The listing builds one solid part. Answer for the finished solid, in the listing's coordinates (mm). A direction names the side the tool comes from. Coordinates: 2 decimals unless noted, no trailing zeros. Write each loop counter-clockwise with the first axis right and the second up, starting at its lowest first coordinate (ties: lowest second). Pieces come first, ordered by that corner, then holes. Notation, with made-up numbers: M 6,31 L 37,31 A16 ccw 37,37 Z; hole C 42.25,89.25 d6. An arc over 180 degrees is marked long. Answer as CSV lines item,"result". Start each with the question number.
```python
from build123d import *


with BuildPart() as part:
    # 草图1 → 旋转1 (revolve)
    with BuildSketch(Plane.XY, mode=Mode.PRIVATE) as revolve_1_sk:
        with BuildLine():
            Line((0, 0), (0, 12.5))
            Line((0, 12.5), (1, 13.5))
            Line((1, 13.5), (41, 13.5))
            Line((41, 13.5), (41, 12.5))
            Line((41, 12.5), (45, 12.5))
            Line((45, 12.5), (45, 13))
            ThreePointArc((45, 13), (45.878679656, 15.121320344), (48, 16))
            Line((48, 16), (711, 16))
            Line((711, 16), (711, 14.5))
            Line((711, 14.5), (713, 14.5))
            Line((713, 14.5), (713, 16))
            Line((713, 16), (718, 16))
            Line((718, 16), (718, 14.5))
            Line((718, 14.5), (720, 14.5))
            Line((720, 14.5), (720, 16))
            Line((720, 16), (724, 16))
            Line((724, 16), (725, 15))
            Line((725, 15), (725, 10))
            Line((725, 10), (754, 10))
            Line((754, 10), (755, 9))
            Line((755, 9), (755, 0))
            Line((755, 0), (0, 0))
        make_face()
    revolve(revolve_1_sk.sketch.rotate(Axis((0, 0, 0), (1, 0, 0)), 90), axis=Axis((0, 0, 0), (1, 0, 0)))


solid = part.part
```
1) For a pull along X with two mould halves and no side action, classify faces 4 (the face through (384.14, 15.62, -3.47)), 5 (the face through (720, -14.3, 3.6)), 6 (the face through (719.014, 12.864, 6.691)), 7 (the face through (725, 10, 3)) as +X half, -X half, draft (parallel to the pull), parting line (faces both ways), or undercut.
2) Find the intervals of material crossed by line 1 (X direction, y = 13.5, z = 8); line 2 (Y direction, x = 393, z = -1); line 3 (X direction, y = -5, z = -10), in increasing order. Write a range as from..to.
3) Each of these flat-tipped pins is pushed along its axis until it touches: P1, Ø4, axis at x = 193, z = -11.5, coming from the -Y side; P2, Ø3, axis at x = 84.5, y = 5, coming from the +Z side; P3, Ø4, axis at x = 267.5, y = 4, coming from the -Z side. Where does it stop, or does it pass through?
4) The part is cut by section A-A (x = 171). Determine the outline of the cut face in (y, z).
5) Which of the six approach directions +Z, -Z, +X, -X, +Y, -Y give full straight-line access (tool end or side, diameter ignored) to faces 1 (the face through (755, 0, 0)), 2 (the face through (740, 0, -10)), 3 (the face through (45, -10.7, 6.8))?
Completed:
1,face 4,"draft"
1,face 5,"undercut"
1,face 6,"undercut"
1,face 7,"+X half"
2,line 1,"46.68..711, 713..718, 720..724.31"
2,line 2,"-15.97..15.97"
2,line 3,"0..725"
3,P1,"y = -12.87"
3,P2,"z = 15.61"
3,P3,"z = -15.87"
4,outline,"C 0,0 d32"
5,face 1,"+Z, -Z, +X, +Y, -Y"
5,face 2,"+X"
5,face 3,"none"
